from build123d import *

# Parameters (mm, degrees)
SKETCH1_R           = 55.5
SKETCH1_R_2         = 44
BOSS_EXTRUDE1_DEPTH = 8
CIRPATTERN1_COUNT   = 4


with BuildPart() as part:
    # Sketch1 → Boss-Extrude1 (new body)
    with BuildSketch(Plane.XY):
        Circle(SKETCH1_R)
        Circle(SKETCH1_R_2, mode=Mode.SUBTRACT)
    extrude(amount=BOSS_EXTRUDE1_DEPTH)

    # Sketch5 → Hole size per socket head cap screw type 1 (revolve, cut)
    with BuildSketch(Plane(origin=(0, 49.5, 8), x_dir=(0, -1, 0), z_dir=(1, 0, 0))):
        Polygon((0, 0), (0, 18.351936393), (2.25, 17), (2.25, 4.6), (4, 4.6), (4, 0), align=None)
    hole_size_per_socket_head_cap_screw_type = revolve(axis=Axis((0, 49.5, 14.35), (0, 0, -1)), mode=Mode.SUBTRACT)

    # CirPattern1: Hole size per socket head cap screw type 1 ×4 about axis
    cirpattern1_axis = Axis((0, 0, 0), (0, 0, 1))
    for i in range(1, CIRPATTERN1_COUNT):
        add(hole_size_per_socket_head_cap_screw_type.rotate(cirpattern1_axis, i * 360 / CIRPATTERN1_COUNT), mode=Mode.SUBTRACT)


solid = part.part
Can you work these out from the model? Positions are in its coordinate system, mm. A direction names the side the tool comes from. Give positions to 0.01 mm unless a question says otherwise; leave off trailing zeros. Order: outer loops, then holes, each group sorted by start corner. A loop starts at its lowest first (then second) coordinate and runs counter-clockwise, first axis right, second up. Notation, with made-up numbers: M 59,40 L 107,40 A15 cw 107,66 Z; hole C 29.25,-33 d11. An arc over 180 degrees is marked long. Use one line per item in the form item = value.
Item 1: If we section it at B-B, the plane z = 1.5: Write out the boundary of the cut face in (x, y).
Values follow:
outline = C 0,0 d111; hole C -49.5,0 d4.5; hole C 0,0 d88; hole C 0,-49.5 d4.5; hole C 0,49.5 d4.5; hole C 49.5,0 d4.5
Item 2: If we section it at C-C, the plane x = -49.5: Write out the boundary of the cut face in (y, z).
Values follow:
outline = M -25.1,0 L -2.25,0 L -2.25,3.4 L -4,3.4 L -4,8 L -25.1,8 Z; M 2.25,0 L 25.1,0 L 25.1,8 L 4,8 L 4,3.4 L 2.25,3.4 Z
Item 3: Will these pins go through, and if not, where does the flat tip stop? pin 1 Ø5 at (x, y) = (0, -49.5) entering from +Z; pin 2 Ø2.5 at (x, y) = (-49.5, 0) entering from +Z (1 decimal); pin 3 Ø3 at (y, z) = (-35.5, 4.5) entering from +X; pin 4 Ø4 at (y, z) = (15.5, 5) entering from -X.
Values follow:
pin_1 = 3.4
pin_2 = through
pin_3 = 43.87
pin_4 = -53.83
Item 4: If I drill on line 1 along Y through (x, z) = (0, 0.9); line 2 along X through (y, z) = (0.5, 7); line 3 along Y through (x, z) = (-31.5, 7.5), over which ranges is the centre line in solid material (lowest first)? Write a range as [from, to].
Values follow:
line_1 = [-55.5, -51.75], [-47.25, -44], [44, 47.25], [51.75, 55.5]
line_2 = [-55.5, -53.47], [-45.53, -44], [44, 45.53], [53.47, 55.5]
line_3 = [-45.69, -30.72], [30.72, 45.69]
Item 5: If we section it at D-D, the plane y = 34.5: Write out the boundary of the cut face in (x, z).
Values follow:
outline = M -43.47,0 L -27.31,0 L -27.31,8 L -43.47,8 Z; M 27.31,0 L 43.47,0 L 43.47,8 L 27.31,8 Z
Item 6: For faces 4 (the cylindrical face through (-53.496, -0.176, 5.732)), 5 (the cylindrical face through (-0.099, 51.748, 1.724)), which set-ups out of +Z, -Z, +X, -X, +Y, -Y let a thin tool reach every point of the face, with its end or its side?
Values follow:
face_4 = +Z
face_5 = +Z, -Z
Item 7: If we section it at A-A, the plane y = -26.5: Write out the boundary of the cut face in (x, z).
Values follow:
outline = M -48.76,0 L -35.12,0 L -35.12,8 L -48.76,8 Z; M 35.12,0 L 48.76,0 L 48.76,8 L 35.12,8 Z
Item 8: Thinking about a two-plate mould opening in X: for faces 1 (the flat face through (-17, 41, 8)), 2 (the cylindrical face through (52.937, 16.671, 3.944)), 3 (the cylindrical face through (0.099, -51.748, 1.724)), which applies, pulls with the +X half, pulls with the -X half, needs draft (parallel to the pull), parting line crosses it, or undercut?
Values follow:
face_1 = needs draft
face_2 = parting line crosses it
face_3 = undercut
